from build123d import *

# Parameters (mm, degrees)
EXTRUDE_1_DEPTH              = 15
HOLE_WIZARD_10_0_10_1_D      = 10
HOLE_WIZARD_8_5_8_5_1_REACH  = 36.989
HOLE_WIZARD_8_5_8_5_1_BORE_R = 4.25
CHAMFER_1_SIZE               = 1


with BuildPart() as part:
    # 草图1 → 凸台-拉伸1 (new body)
    with BuildSketch(Plane.XY.offset(7.5)):
        with BuildLine():
            Line((7.5, 20), (-7.5, 20))
            Line((-7.5, 20), (-7.5, 9.367496998))
            ThreePointArc((-7.5, 9.367496998), (0, -12), (7.5, 9.367496998))
            Line((7.5, 9.367496998), (7.5, 20))
        make_face()
    extrude(amount=-EXTRUDE_1_DEPTH)

    # Ø10.0 (10) 直径孔1 (through all)
    with Locations(Plane.XY.offset(7.5)):
        with Locations((0, 0)):
            Hole(HOLE_WIZARD_10_0_10_1_D / 2)

    # Ø8.5 (8.5) 直径孔1 bore → Ø8.5 (8.5) 直径孔1 (cut, up to next)
    with BuildSketch(Plane(origin=(0, 20, 0), x_dir=(1, 0, 0), z_dir=(0, 1, 0)), mode=Mode.PRIVATE) as hole_wizard_8_5_8_5_1_sk1:
        Circle(HOLE_WIZARD_8_5_8_5_1_BORE_R)
    hole_wizard_8_5_8_5_1_tool1 = extrude(hole_wizard_8_5_8_5_1_sk1.sketch, amount=-HOLE_WIZARD_8_5_8_5_1_REACH, mode=Mode.PRIVATE) & part.part
    add(hole_wizard_8_5_8_5_1_tool1.solids().sort_by_distance((0, 20, 0))[0], mode=Mode.SUBTRACT)

    # 倒角1
    chamfer_1_edges = [part.edges().sort_by_distance(p)[0] for p in [
        (-7.5, 14.683748499, -7.5),
        (0, -12, -7.5),
        (7.5, 14.683748499, -7.5),
        (0, -12, 7.5),
        (-7.5, 14.683748499, 7.5),
        (7.5, 14.683748499, 7.5),
    ]]
    chamfer(chamfer_1_edges, length=CHAMFER_1_SIZE)


solid = part.part
CAD build for the part. Positions are in the model's coordinates, mm. A direction names the side the tool comes from. Give positions to 0.01 mm unless a question says otherwise; leave off trailing zeros. Write each loop counter-clockwise with the first axis right and the second up, starting at its lowest first coordinate (ties: lowest second). Pieces come first, ordered by that corner, then holes. Notation, with made-up numbers: M 49.5,34 L 63.5,34 A10 ccw 63.5,42 Z; hole C 51.25,42 d11. An arc over 180 degrees is marked long. Put each result on its own line as item: value. Start each with the question number.
(1) Mould opens along Y. For faces 1 (the face through (-0.392, -11.167, -7.326)), 2 (the face through (3.4, 20, 3.4)), 3 (the face through (1.08, -4.88, -0.1)) say: +Y half, -Y half, draft (parallel to the pull), parting line (faces both ways), or undercut.
(2) Flat gauge pins, fed straight in: pin 1 Ø6 at (x, z) = (-3.5, 1.5) entering from -Y; pin 2 Ø3 at (y, z) = (13, -3) entering from -X; pin 3 Ø6 at (y, z) = (5, 5) entering from +X; pin 4 Ø1.5 at (x, y) = (-9, 12.5) entering from +Z. Where does each tip first touch, or does it go through?
(3) Which spindle directions (+Z, -Z, +X, -X, +Y, -Y) get a long thin tool onto all of the face, cutting with end or side? Do faces 4 (the face through (-0.92, 11.44, 4.15)), 5 (the face through (7.5, 15, 0)), 6 (the face through (-7, 15, -7)), 7 (the face through (7, 14, 7)), 8 (the face through (-7, 15, 7)). Say none if no direction does.
(4) Band-saw the part on A-A, the plane y = 13.5. Write the cut outline in (x, z).
(5) Band-saw the part on B-B, the plane x = 0. Write the cut outline in (y, z).
(6) Probe L1, parallel to X at y = 13, z = 0; L2, parallel to Y at x = 0, z = 4. List the from-to ranges inside material, lowest first.
(7) Band-saw the part on C-C, the plane z = 0. Write the cut outline in (x, y), and give its area (3 significant figures).
(8) Band-saw the part on D-D, the plane x = -3. Give the number of separate pieces and of enclosed holes in the cut face, and give its area (3 significant figures).
Response values:
1. face 1: parting line
1. face 2: +Y half
1. face 3: undercut
2. pin 1: stops at y = -11.99
2. pin 2: stops at x = -7.5
2. pin 3: stops at x = 11.83
2. pin 4: passes through
3. face 4: +Y
3. face 5: +Z, -Z, +X, +Y
3. face 6: -Z, -X, +Y
3. face 7: +Z, +X, +Y
3. face 8: +Z, -X, +Y
4. outline: M -7.5,-6.5 L -6.5,-7.5 L 6.5,-7.5 L 7.5,-6.5 L 7.5,6.5 L 6.5,7.5 L -6.5,7.5 L -7.5,6.5 Z; hole C 0,0 d8.5
5. outline: M -12,-6.5 L -11,-7.5 L -5,-7.5 L -5,7.5 L -11,7.5 L -12,6.5 Z; M 5,-7.5 L 20,-7.5 L 20,-4.25 L 5,-4.25 Z; M 5,4.25 L 20,4.25 L 20,7.5 L 5,7.5 Z
6. L1: x = -7.5 to -4.25, 4.25 to 7.5
6. L2: y = -12 to -5
7. outline: M -7.5,9.37 A12 ccw long 7.5,9.37 L 7.5,20 L 4.25,20 L 4.25,2.63 A5 cw long -4.25,2.63 L -4.25,20 L -7.5,20 Z
7. area: 373 mm2
8. separate pieces: 3
8. enclosed holes: 0
8. area: 257 mm2
